Verification items for the finished model (mm, model axes). Face numbers are marked on the shaded views. A direction names the side the tool comes from. Give positions to 0.01 mm unless a question says otherwise; leave off trailing zeros. Order: outer loops, then holes, each group sorted by start corner. A loop starts at its lowest first (then second) coordinate and runs counter-clockwise, first axis right, second up. Notation, with made-up numbers: (85.5, 42) - (124.5, 42) arc R33 ccw to (124.5, 71) - close; hole circle Ø3 at (46, -18.75). An arc over 180 degrees is marked (long way). Answer as a JSON object with one key per item and string values. Group by question number.
(1) Depth check by flat-ended pin: pin 1 Ø6.5 at (y, z) = (44.5, 0) entering from +X; pin 2 Ø9 at (y, z) = (45, -2) entering from -X; pin 3 Ø10 at (x, z) = (7.5, -16) entering from +Y; pin 4 Ø19 at (x, z) = (4, -2) entering from -Y. Enter the tip coordinate at first touch or a pass-through.
(2) Access from +Z, -Z, +X, -X, +Y, -Y to the whole of each face (thin tool, end or side, straight path). Record for the marked faces 1 and 2.
(3) Section check A-A (z = 0). Record the boundary of the cut face in (x, y).
(4) Section check B-B (y = 33). Record the boundary of the cut face in (x, z), then the cut area to 3 significant figures.
(5) Thickness scan on line 1 (Y direction, x = -5, z = 7.5); line 2 (Y direction, x = -6, z = 12.5); line 3 (Z direction, x = 0.5, y = 52). Record the ranges inside material, lowest first.
```python
from build123d import *

# Parameters (mm, degrees)
SKETCH_2_R      = 8
EXTRUDE_1_DEPTH = 10
EXTRUDE_2_DEPTH = 8
SKETCH_4_R      = 10
EXTRUDE_3_DEPTH = 120


with BuildPart() as part:
    # 草图1 → 旋转1 (revolve)
    with BuildSketch(Plane.XY, mode=Mode.PRIVATE) as revolve_1_sk:
        Polygon((0, 30), (0, 0), (50, 0), (50, 10), (15, 30), align=None)
    revolve(revolve_1_sk.sketch.rotate(Axis((0, 30, 0), (0, -1, 0)), 180), axis=Axis((0, 30, 0), (0, -1, 0)))

    # 草图2 → 凸台-拉伸1 (add)
    with BuildSketch(Plane(origin=(0, 30, 0), x_dir=(1, 0, 0), z_dir=(0, 1, 0))):
        Circle(SKETCH_2_R)
    extrude(amount=EXTRUDE_1_DEPTH)

    # 草图3 → 凸台-拉伸2 (add)
    with BuildSketch(Plane(origin=(0, 40, 0), x_dir=(1, 0, 0), z_dir=(0, 1, 0))):
        Polygon((0, 13.856406461), (-12, 6.92820323), (-12, -6.92820323), (0, -13.856406461), (12, -6.92820323), (12, 6.92820323), align=None)
    extrude(amount=EXTRUDE_2_DEPTH)

    # 草图4 → 凸台-拉伸3 (add)
    with BuildSketch(Plane(origin=(0, 48, 0), x_dir=(1, 0, 0), z_dir=(0, 1, 0))):
        with Locations(Location((0, 0, 0), (0, 0, 270))):
            Circle(SKETCH_4_R)
    extrude(amount=EXTRUDE_3_DEPTH)


solid = part.part
```
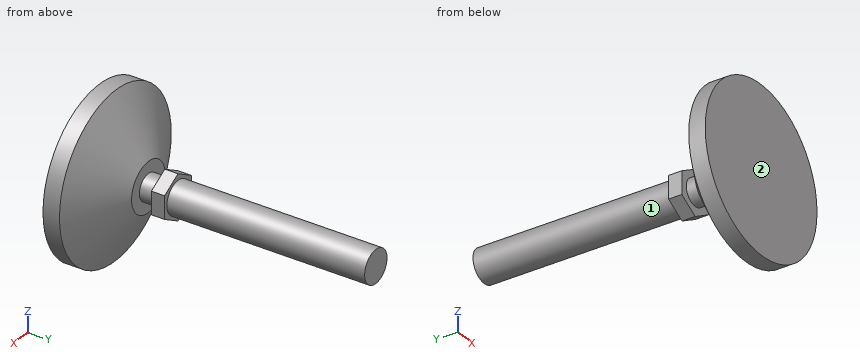
Solutions:
{
 "1": {"pin 1": "stops at x = 12", "pin 2": "stops at x = -12", "pin 3": "stops at y = 30", "pin 4": "stops at y = 0"},
 "2": {"face 1": "+Y", "face 2": "+Z, -Z, +X, -X, -Y"},
 "3": {"outline": "(-50, 0) - (50, 0) - (50, 10) - (15, 30) - (8, 30) - (8, 40) - (12, 40) - (12, 48) - (10, 48) - (10, 168) - (-10, 168) - (-10, 48) - (-12, 48) - (-12, 40) - (-8, 40) - (-8, 30) - (-15, 30) - (-50, 10) - close"},
 "4": {"outline": "circle Ø16 at (0, 0)", "area": "201 mm2"},
 "5": {"line 1": "y = 0 to 30, 40 to 168", "line 2": "y = 0 to 30", "line 3": "z = -9.99 to 9.99"}
}
